```python
from build123d import *

# Parameters (mm, degrees)
EXTRUDE_1_DEPTH              = 15
CHAMFER_1_SIZE               = 0.5
HOLE_WIZARD_M3_1_D           = 3.4
HOLE_WIZARD_M3_1_DEPTH       = 10
HOLE_WIZARD_M3_1_CBORE_D     = 6.5
HOLE_WIZARD_M3_1_CBORE_DEPTH = 3.4
HOLE_WIZARD_M3_1_TIP         = 1.021463052


with BuildPart() as part:
    # 草图2 → 凸台-拉伸1 (new body)
    with BuildSketch(Plane.ZY.offset(7.5)):
        with BuildLine():
            Line((-6, -6.8), (-8, -6.8))
            Line((-8, -6.8), (-8, -8.2))
            Line((-8, -8.2), (-2, -8.2))
            Line((-2, -8.2), (-0.741180955, -7.862700453))
            ThreePointArc((-0.741180955, -7.862700453), (-0.20664666, -7.505536056), (0, -6.896774627))
            Line((0, -6.896774627), (0, 6.896774627))
            ThreePointArc((0, 6.896774627), (-0.20664666, 7.505536056), (-0.741180955, 7.862700453))
            Line((-0.741180955, 7.862700453), (-2, 8.2))
            Line((-2, 8.2), (-8, 8.2))
            Line((-8, 8.2), (-8, 7.7))
            Line((-8, 7.7), (-8, 6.8))
            Line((-8, 6.8), (-6, 6.8))
            Line((-6, 6.8), (-6, -6.8))
        make_face()
    extrude(amount=-EXTRUDE_1_DEPTH)

    # 倒角1
    chamfer_1_edges = [part.edges().sort_by_distance(p)[0] for p in [
        (-7.5, 8.2, -5),
        (-7.5, 8.031350227, -1.370590477),
        (-7.5, 7.505536056, -0.20664666),
        (-7.5, 0, 0),
        (-7.5, -7.505536056, -0.20664666),
        (-7.5, -8.031350227, -1.370590477),
        (-7.5, -8.2, -5),
        (7.5, -8.2, -5),
        (7.5, -8.031350227, -1.370590477),
        (7.5, -7.505536056, -0.20664666),
        (7.5, 0, 0),
        (7.5, 7.505536056, -0.20664666),
        (7.5, 8.031350227, -1.370590477),
        (7.5, 8.2, -5),
    ]]
    chamfer(chamfer_1_edges, length=CHAMFER_1_SIZE)

    # M3 六角凹头螺钉的柱形沉头孔1
    with Locations(Plane.XY):
        with Locations((0, 0)):
            CounterBoreHole(HOLE_WIZARD_M3_1_D / 2, HOLE_WIZARD_M3_1_CBORE_D / 2, HOLE_WIZARD_M3_1_CBORE_DEPTH, depth=HOLE_WIZARD_M3_1_DEPTH)
            with Locations((0, 0, -(HOLE_WIZARD_M3_1_DEPTH + HOLE_WIZARD_M3_1_TIP / 2))):  # 118° drill point
                Cone(0, HOLE_WIZARD_M3_1_D / 2, HOLE_WIZARD_M3_1_TIP, mode=Mode.SUBTRACT)


solid = part.part
```
Can you work these out from the model? Positions are in its coordinate system, mm. A direction names the side the tool comes from. Coordinates: 2 decimals unless noted, no trailing zeros. Loops run counter-clockwise (first coordinate to the right, second up) from the corner with the lowest first, then second, coordinate; pieces in that order, holes last. Notation, with made-up numbers: (-36, 87.25) - (12, 87.25) arc R22 ccw to (12, 124.25) - close; hole circle Ø10 at (47, 83.25). An arc over 180 degrees is marked (long way). Answer as CSV lines item,"result". Start each with the question number.
1) Which directions (+Z, -Z, +X, -X, +Y, -Y) give clear straight access to the entire face, cutting with the end or side of a thin tool? Please do faces 1 (the cylindrical face through (-2.579, -1.978, -1.676)), 2 (the conical face through (7.25, -7.36, -0.41)), 3 (the flat face through (0, 6.8, -7)).
2) Suppose I cut it at A-A (y = 0). Please give me the cut outline in (x, z).
3) Suppose I cut it at C-C (x = 0). Please give me the cut outline in (y, z).
4) For pin 1 (8 mm diameter, centred on x = 5.5, y = 4.5, fed in from -Z); pin 2 (1.5 mm diameter, centred on x = 0, y = 1, fed in from +Z); pin 3 (2.5 mm diameter, centred on x = 0, y = 0, fed in from +Z); pin 4 (4 mm diameter, centred on x = 0, y = 0, fed in from -Z), each with a flat end and sliding along its axis, tell me the tip position at first contact or that it passes through.
5) I need wall thicknesses on line 1 (Y direction, x = 0, z = -5.2); line 2 (Z direction, x = -3.5, y = 1); line 3 (Y direction, x = 1.25, z = -5). Which ranges of each line are inside material? Lowest first, please. Write a range as from..to.
6) Thinking about a two-plate mould opening in Y: for faces 4 (the cylindrical face through (-0.1, -7.5, -0.2)), 5 (the flat face through (1.4, -1.4, -3.4)), 6 (the flat face through (0, 8.2, -5)), which applies, pulls with the +Y half, pulls with the -Y half, needs draft (parallel to the pull), parting line crosses it, or undercut?
7) Suppose I cut it at B-B (z = -7). Please give me the cut outline in (x, y).
8) Suppose I cut it at D-D (z = -4.75). Please give me the cut outline in (x, y).
Check result:
1,face 1,"+Z"
1,face 2,"+Z, +X, -Y"
1,face 3,"-Z, +X, -X"
2,outline,"(-7.5, -6) - (-1.7, -6) - (-1.7, -3.4) - (-3.25, -3.4) - (-3.25, 0) - (-7, 0) - (-7.5, -0.5) - close; (1.7, -6) - (7.5, -6) - (7.5, -0.5) - (7, 0) - (3.25, 0) - (3.25, -3.4) - (1.7, -3.4) - close"
3,outline,"(-8.2, -8) - (-6.8, -8) - (-6.8, -6) - (-1.7, -6) - (-1.7, -3.4) - (-3.25, -3.4) - (-3.25, 0) - (-6.9, 0) arc R1 ccw to (-7.86, -0.74) - (-8.2, -2) - close; (1.7, -6) - (6.8, -6) - (6.8, -8) - (8.2, -8) - (8.2, -2) - (7.86, -0.74) arc R1 ccw to (6.9, 0) - (3.25, 0) - (3.25, -3.4) - (1.7, -3.4) - close"
4,pin 1,"stops at z = -8"
4,pin 2,"stops at z = -3.4"
4,pin 3,"passes through"
4,pin 4,"stops at z = -6"
5,line 1,"y = -8.2..-1.7, 1.7..8.2"
5,line 2,"z = -6..0"
5,line 3,"y = -8.2..-1.15, 1.15..8.2"
6,face 4,"pulls with the -Y half"
6,face 5,"undercut"
6,face 6,"pulls with the +Y half"
7,outline,"(-7.5, -7.7) - (-7, -8.2) - (7, -8.2) - (7.5, -7.7) - (7.5, -6.8) - (-7.5, -6.8) - close; (-7.5, 6.8) - (7.5, 6.8) - (7.5, 7.7) - (7, 8.2) - (-7, 8.2) - (-7.5, 7.7) - close"
8,outline,"(-7.5, -7.7) - (-7, -8.2) - (7, -8.2) - (7.5, -7.7) - (7.5, 7.7) - (7, 8.2) - (-7, 8.2) - (-7.5, 7.7) - close; hole circle Ø3.4 at (0, 0)"
